Could you check a few things on this model? Use its own coordinates, in mm. Round coordinates to 2 decimals unless told otherwise and drop trailing zeros. Loops run counter-clockwise (first coordinate to the right, second up) from the corner with the lowest first, then second, coordinate; pieces in that order, holes last. Notation, with made-up numbers: (72.5, 42) - (78.5, 42) arc R28 cw to (78.5, 65) - close; hole circle Ø7 at (1, 45). An arc over 180 degrees is marked (long way). Put each result on its own line as item: value. Start each with the question number.
from build123d import *

# Parameters (mm, degrees)
SKETCH1_R           = 7
BOSS_EXTRUDE1_DEPTH = 2.5


with BuildPart() as part:
    # Sketch1 → Boss-Extrude1 (new, symmetric)
    with BuildSketch(Plane.XY):
        with BuildLine():
            Line((20, 0), (-20, 0))
            Line((-20, 0), (-12.57432219, 28.299457752))
            ThreePointArc((-12.57432219, 28.299457752), (0, 38), (12.57432219, 28.299457752))
            Line((12.57432219, 28.299457752), (20, 0))
        make_face()
        with Locations((0, 25)):
            Circle(SKETCH1_R, mode=Mode.SUBTRACT)
    extrude(amount=BOSS_EXTRUDE1_DEPTH, both=True)


solid = part.part
Item 1: Suppose I cut it at D-D, the plane y = 9.5. List the corners of the cut face in (x, z) for me, then the cut area to 3 significant figures.
Item 2: I need wall thicknesses on line 1 (X direction, y = 20, z = 1.75); line 2 (Y direction, x = -3, z = -0.6); line 3 (X direction, y = 25.5, z = 2). Which ranges of each line are inside material? Lowest first, please. Write a range as from..to.
Item 3: Suppose I cut it at C-C, the plane z = -1. List the corners of the cut face in (x, y) for me, then the cut area to 3 significant figures.
Item 4: Will these pins go through, and if not, where does the flat tip stop? P1, Ø1, axis at y = 16, z = -0.5, coming from the -X side; P2, Ø1.5, axis at y = 20.5, z = 1, coming from the -X side.
Item 5: Suppose I cut it at A-A, the plane x = 0. List the corners of the cut face in (y, z) for me, then the cut area to 3 significant figures.
Item 6: Thinking about a two-plate mould opening in Y: for faces 1 (the face through (-1.517, 18.166, -0.035)), 2 (the face through (16.235, 14.348, 0.035)), 3 (the face through (0, 0, 0)), which applies, released by +Y, released by -Y, zero draft, split by the parting line, or undercut?
Item 7: Suppose I cut it at B-B, the plane y = 30. List the corners of the cut face in (x, z) for me, then the cut area to 3 significant figures.
Numbers:
1. outline: (-17.51, -2.5) - (17.51, -2.5) - (17.51, 2.5) - (-17.51, 2.5) - close
1. area: 175 mm^2
2. line 1: -14.75..-4.9, 4.9..14.75
2. line 2: 0..18.68, 31.32..37.65
2. line 3: -13.31..-6.98, 6.98..13.31
3. outline: (-20, 0) - (20, 0) - (12.57, 28.3) arc R13 ccw to (-12.57, 28.3) - close; hole circle Ø14 at (0, 25)
3. area: 949 mm^2
4. P1: x = -15.93
4. P2: x = -14.82
5. outline: (0, -2.5) - (18, -2.5) - (18, 2.5) - (0, 2.5) - close; (32, -2.5) - (38, -2.5) - (38, 2.5) - (32, 2.5) - close
5. area: 120 mm^2
6. face 1: undercut
6. face 2: released by +Y
6. face 3: released by -Y
7. outline: (-12, -2.5) - (-4.9, -2.5) - (-4.9, 2.5) - (-12, 2.5) - close; (4.9, -2.5) - (12, -2.5) - (12, 2.5) - (4.9, 2.5) - close
7. area: 71.0 mm^2
